from build123d import *

# Parameters (mm, degrees)
CHAMFER1_SIZE = 1


with BuildPart() as part:
    # Sketch1 → Revolve1 (revolve)
    with BuildSketch(Plane(origin=(0, 0, 0), x_dir=(0, 0, -1), z_dir=(1, 0, 0)), mode=Mode.PRIVATE) as revolve1_sk:
        Polygon((15, 0), (15, 12.5), (10, 12.5), (10, 9.05), (0, 9.05), (0, 0), align=None)
    revolve(revolve1_sk.sketch.rotate(Axis((0, 0, 0), (0, 0, -1)), 90), axis=Axis((0, 0, 0), (0, 0, -1)))

    # Chamfer1
    chamfer1_edges = [part.edges().sort_by_distance(p)[0] for p in [
        (-9.05, 0, 0),
        (-12.5, 0, -10),
        (-12.5, 0, -15),
    ]]
    chamfer(chamfer1_edges, length=CHAMFER1_SIZE)


solid = part.part
Can you work these out from the model? Positions are in its coordinate system, mm. A direction names the side the tool comes from. Round coordinates to 2 decimals unless told otherwise and drop trailing zeros. Write each loop counter-clockwise with the first axis right and the second up, starting at its lowest first coordinate (ties: lowest second). Pieces come first, ordered by that corner, then holes. Notation, with made-up numbers: (-1, 40.25) -> (34, 40.25) arc R8 ccw to (34, 55.25) -> close; hole circle Ø5 at (29.5, -18). An arc over 180 degrees is marked (long way). Use one line per item in the form item = value. Start each with the question number.
Q1. Which directions (+Z, -Z, +X, -X, +Y, -Y) give clear straight access to the entire face, cutting with the end or side of a thin tool? Please do faces 1 (the face through (11.923, -3.755, -12.479)), 2 (the face through (8.63, -2.72, -5.44)).
Q2. Imagine slicing it at D-D (z = -12). Please give me the cut outline in (x, y).
Q3. I'm going to push flat-ended pins straight in: P1, Ø3, axis at x = -1.5, z = -12.5, coming from the +Y side; P2, Ø1.5, axis at x = 1, z = -5, coming from the -Y side; P3, Ø6, axis at y = 6.5, z = -8, coming from the +X side; P4, Ø5, axis at x = -4, z = -3, coming from the +Y side. Where does each tip first touch, or does it pass through?
Q4. If I drill on probe 1 along Z at (x, y) = (-6.5, -7.25); probe 2 along Y at (x, z) = (0.25, -1.5); probe 3 along Y at (x, z) = (6.25, -4.5), over which ranges is the centre line in solid material (lowest first)? Write a range as [from, to].
Q5. Imagine slicing it at C-C (z = -3.75). Please give me the cut outline in (x, y), then the cut area to 3 significant figures.
Q6. Imagine slicing it at A-A (y = 0). Please give me the cut outline in (x, z).
Worked out:
q1.face_1 = +Z, -Z
q1.face_2 = +Z
q2.outline = circle Ø25 at (0, 0)
q3.P1 = 12.5
q3.P2 = -9.05
q3.P3 = 11.04
q3.P4 = 8.92
q4.probe_1 = [-15, -10]
q4.probe_2 = [-9.05, 9.05]
q4.probe_3 = [-6.55, 6.55]
q5.outline = circle Ø18.1 at (0, 0)
q5.area = 257 mm^2
q6.outline = (-12.5, -14) -> (-11.5, -15) -> (11.5, -15) -> (12.5, -14) -> (12.5, -11) -> (11.5, -10) -> (9.05, -10) -> (9.05, -1) -> (8.05, 0) -> (-8.05, 0) -> (-9.05, -1) -> (-9.05, -10) -> (-11.5, -10) -> (-12.5, -11) -> close
